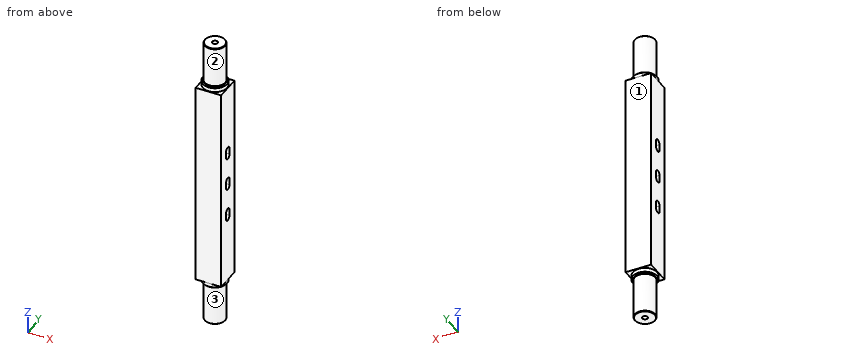
from build123d import *

# Parameters (mm, degrees)
SKETCH_1_R              = 20
EXTRUDE_1_DEPTH         = 79
SKETCH_2_R              = 23.75
EXTRUDE_2_DEPTH         = 10
CHAMFER_1_SIZE          = 2
SKETCH_3_W              = 50
SKETCH_3_H              = 50
EXTRUDE_3_DEPTH         = 406.5
SKETCH_4_R              = 23.75
EXTRUDE_4_DEPTH         = 10
CHAMFER_2_SIZE          = 2
SKETCH_5_R              = 20
EXTRUDE_5_DEPTH         = 79
CHAMFER_3_SIZE          = 1
HOLE_WIZARD_M12_1_D     = 10.2
HOLE_WIZARD_M12_1_DEPTH = 29.25
HOLE_WIZARD_M12_1_TIP   = 3.064389157
HOLE_WIZARD_M12_2_D     = 10.2
HOLE_WIZARD_M12_2_DEPTH = 29.25
HOLE_WIZARD_M12_2_TIP   = 3.064389157
CUT_EXTRUDE_1_DEPTH     = 79


with BuildPart() as part:
    # 草图1 → 凸台-拉伸1 (new body)
    with BuildSketch(Plane.XY):
        Circle(SKETCH_1_R)
    extrude(amount=EXTRUDE_1_DEPTH)

    # 草图2 → 凸台-拉伸2 (add)
    with BuildSketch(Plane.XY.offset(79)):
        Circle(SKETCH_2_R)
    extrude(amount=EXTRUDE_2_DEPTH)

    # 倒角1
    chamfer_1_edges = [part.edges().sort_by_distance(p)[0] for p in [
        (-23.75, 0, 79),
    ]]
    chamfer(chamfer_1_edges, length=CHAMFER_1_SIZE)

    # 草图3 → 凸台-拉伸3 (add)
    with BuildSketch(Plane.XY.offset(89)):
        Rectangle(SKETCH_3_W, SKETCH_3_H)
    extrude(amount=EXTRUDE_3_DEPTH)

    # 草图4 → 凸台-拉伸4 (add)
    with BuildSketch(Plane.XY.offset(495.5)):
        Circle(SKETCH_4_R)
    extrude(amount=EXTRUDE_4_DEPTH)

    # 倒角2
    chamfer_2_edges = [part.edges().sort_by_distance(p)[0] for p in [
        (-23.75, 0, 505.5),
    ]]
    chamfer(chamfer_2_edges, length=CHAMFER_2_SIZE)

    # 草图5 → 凸台-拉伸5 (add)
    with BuildSketch(Plane.XY.offset(505.5)):
        Circle(SKETCH_5_R)
    extrude(amount=EXTRUDE_5_DEPTH)

    # 倒角3
    chamfer_3_edges = [part.edges().sort_by_distance(p)[0] for p in [
        (-20, 0, 0),
        (-20, 0, 584.5),
    ]]
    chamfer(chamfer_3_edges, length=CHAMFER_3_SIZE)

    # M12 螺纹孔1
    with Locations(Plane(origin=(0, 0, 0), x_dir=(-1, 0, 0), z_dir=(0, 0, -1))):
        with Locations((0, 0)):
            Hole(HOLE_WIZARD_M12_1_D / 2, depth=HOLE_WIZARD_M12_1_DEPTH)
            with Locations((0, 0, -(HOLE_WIZARD_M12_1_DEPTH + HOLE_WIZARD_M12_1_TIP / 2))):  # 118° drill point
                Cone(0, HOLE_WIZARD_M12_1_D / 2, HOLE_WIZARD_M12_1_TIP, mode=Mode.SUBTRACT)

    # M12 螺纹孔2
    with Locations(Plane.XY.offset(584.5)):
        with Locations((0, 0)):
            Hole(HOLE_WIZARD_M12_2_D / 2, depth=HOLE_WIZARD_M12_2_DEPTH)
            with Locations((0, 0, -(HOLE_WIZARD_M12_2_DEPTH + HOLE_WIZARD_M12_2_TIP / 2))):  # 118° drill point
                Cone(0, HOLE_WIZARD_M12_2_D / 2, HOLE_WIZARD_M12_2_TIP, mode=Mode.SUBTRACT)

    # 草图10 → 切除-拉伸1 (cut)
    with BuildSketch(Plane(origin=(25, 0, 0), x_dir=(0, 0, -1), z_dir=(1, 0, 0))):
        with BuildLine():
            Line((-363.25, 6.5), (-351.25, 6.5))
            ThreePointArc((-351.25, 6.5), (-344.75, 0), (-351.25, -6.5))
            Line((-351.25, -6.5), (-363.25, -6.5))
            ThreePointArc((-363.25, -6.5), (-369.75, 0), (-363.25, 6.5))
        make_face()
        with BuildLine():
            Line((-298.25, 6.5), (-286.25, 6.5))
            ThreePointArc((-286.25, 6.5), (-279.75, 0), (-286.25, -6.5))
            Line((-286.25, -6.5), (-298.25, -6.5))
            ThreePointArc((-298.25, -6.5), (-304.75, 0), (-298.25, 6.5))
        make_face()
        with BuildLine():
            Line((-233.25, 6.5), (-221.25, 6.5))
            ThreePointArc((-221.25, 6.5), (-214.75, 0), (-221.25, -6.5))
            Line((-221.25, -6.5), (-233.25, -6.5))
            ThreePointArc((-233.25, -6.5), (-239.75, 0), (-233.25, 6.5))
        make_face()
    extrude(amount=-CUT_EXTRUDE_1_DEPTH, mode=Mode.SUBTRACT)


solid = part.part
Can you work these out from the model? Positions are in its coordinate system, mm. Face numbers are marked on the shaded views. A direction names the side the tool comes from. Coordinates: 2 decimals unless noted, no trailing zeros. Use one line per item in the form item = value.
Q1. Which directions (+Z, -Z, +X, -X, +Y, -Y) give clear straight access to the entire face, cutting with the end or side of a thin tool? Please do the marked faces 1, 2 and 3.
From the geometry:
face_1 = +Z, -Z, +X, -X, +Y
face_2 = +Z
face_3 = -Z
Q2. Imagine slicing it at A-A, the plane x = -10. Give the number of separate pieces and of enclosed holes in the cut face, then the cut area to 3 significant figures.
From the geometry:
separate_pieces = 1
enclosed_holes = 3
area = 25,800 mm²
Q3. I need wall thicknesses on L1, parallel to Z at x = 13, y = -0.5; L2, parallel to Y at x = -3, z = 298; L3, parallel to Y at x = 0, z = 567.5. Which ranges of each line are inside material? Lowest first, please.
From the geometry:
L1 = 0 to 214.77, 239.73 to 279.77, 304.73 to 344.77, 369.73 to 584.5
L2 = -25 to -6.5, 6.5 to 25
L3 = -20 to -5.1, 5.1 to 20
Q4. Will this pin go through, and if not, where does the flat tip stop? P1, Ø12, axis at y = 7, z = 62, coming from the +X side (3 decimals).
From the geometry:
P1 = 19.975
